Geometry: final body of the model. Coordinates: model frame, mm. A direction names the side the tool comes from. Coordinates: 2 decimals unless noted, no trailing zeros. Order: outer loops, then holes, each group sorted by start corner. A loop starts at its lowest first (then second) coordinate and runs counter-clockwise, first axis right, second up. Notation, with made-up numbers: (-9, 85.5) -> (13, 85.5) arc R23 cw to (13, 123.5) -> close; hole circle Ø8 at (79, 15.25). An arc over 180 degrees is marked (long way). Answer in a Markdown table with one row per item. Add a question column.
1) Section query C-C on x = -194. Return the cut outline in (y, z), then the cut area to 3 significant figures.
2) Contact query for flat-ended pins moving along their axis: P1, Ø4, axis at y = 8.5, z = -590, coming from the +X side; P2, Ø1, axis at x = -167, y = -36.5, coming from the -Z side; P3, Ø8, axis at x = 11.5, z = -937.5, coming from the -Y side. Output: stop coordinate, or through.
3) Section query A-A on y = 0. Return the cut outline in (x, z), then the cut area to 3 significant figures.
4) Pull-direction query (Y, two-part tool) for faces 4 (the face through (44.83, -14.12, -603.33)), 5 (the face through (-188.72, -15.02, -1337.69)), 6 (the face through (-34, -33, 0)); classes: +Y half, -Y half, draft (parallel to the pull), parting line (faces both ways), or undercut.
5) Set-up query: faces 1 (the face through (47.69, -15.02, -603.33)), 2 (the face through (-188.725, -2.067, -1243.045)), 3 (the face through (-275, 33, -1324)). Return all of +Z, -Z, +X, -X, +Y, -Y with unobstructed straight access to the full face (end or side cutting, diameter ignored); none if empty.
6) Ray query, line 1 (Y direction, x = 0, z = -433.5); line 2 (Z direction, x = -174, y = 0). Return the intervals inside material, ascending. Write a range as from..to.
7) Section query B-B on z = -689. Return the cut outline in (x, y), then the cut area to 3 significant figures.
```python
from build123d import *

# Parameters (mm, degrees)
SKETCH_1_R = 50
SHELL_1_T  = -3


with BuildPart() as part:
    # 扫描1: sweep along a path in 草图2
    with BuildLine(Plane(origin=(0, 0, 0), x_dir=(1, 0, 0), z_dir=(0, 1, 0))) as sweep_1_path:
        Line((0, 0), (0, 1190))
        ThreePointArc((0, 1190), (-29.289321881, 1260.710678119), (-100, 1290))
        Line((-100, 1290), (-275, 1290))
    # 草图1 → 扫描1 (sweep)
    with BuildSketch(Plane.XY):
        Circle(SKETCH_1_R)
    sweep(path=sweep_1_path.line)

    # 抽壳1
    shell_1_openings = [part.faces().sort_by_distance(p)[0] for p in [
        (-275, 0, -1290),
        (0, 0, 0),
    ]]
    offset(amount=SHELL_1_T, openings=shell_1_openings, kind=Kind.INTERSECTION)


solid = part.part
```
Result:
| question | item | result |
|---|---|---|
| 1 | outline | circle Ø100 at (0, -1290); hole circle Ø94 at (0, -1290) |
| 1 | area | 914 mm2 |
| 2 | P1 | x = 49.58 |
| 2 | P2 | z = -1324.7 |
| 2 | P3 | y = -49.43 |
| 3 | outline | (-275, -1340) -> (-100, -1340) arc R150 ccw to (50, -1190) -> (50, 0) -> (47, 0) -> (47, -1190) arc R147 cw to (-100, -1337) -> (-275, -1337) -> close; (-275, -1243) -> (-100, -1243) arc R53 ccw to (-47, -1190) -> (-47, 0) -> (-50, 0) -> (-50, -1190) arc R50 cw to (-100, -1240) -> (-275, -1240) -> close |
| 3 | area | 9,130 mm2 |
| 4 | face 4 | undercut |
| 4 | face 5 | parting line |
| 4 | face 6 | draft |
| 5 | face 1 | +Z |
| 5 | face 2 | -X |
| 5 | face 3 | +Z, -Z, -X, +Y, -Y |
| 6 | line 1 | -50..-47, 47..50 |
| 6 | line 2 | -1340..-1337, -1243..-1240 |
| 7 | outline | circle Ø100 at (0, 0); hole circle Ø94 at (0, 0) |
| 7 | area | 914 mm2 |
